from build123d import *

# Parameters (mm, degrees)
SKETCH1_W           = 110
SKETCH1_H           = 70
BOSS_EXTRUDE1_DEPTH = 1
SKETCH2_R           = 5.5
CUT_EXTRUDE1_DEPTH  = 1
CHAMFER1_SIZE       = 5


with BuildPart() as part:
    # Sketch1 → Boss-Extrude1 (new body)
    with BuildSketch(Plane.XY):
        Rectangle(SKETCH1_W, SKETCH1_H)
    extrude(amount=BOSS_EXTRUDE1_DEPTH)

    # Sketch2 → Cut-Extrude1 (cut)
    with BuildSketch(Plane.XY.offset(1)):
        with Locations((-40, 20)):
            Circle(SKETCH2_R)
        with Locations((40, 20)):
            Circle(SKETCH2_R)
        with Locations((-40, -20)):
            Circle(SKETCH2_R)
        with Locations((40, -20)):
            Circle(SKETCH2_R)
    extrude(amount=-CUT_EXTRUDE1_DEPTH, mode=Mode.SUBTRACT)

    # Chamfer1
    chamfer1_edges = [part.edges().sort_by_distance(p)[0] for p in [
        (-55, 35, 0.5),
        (55, 35, 0.5),
        (55, -35, 0.5),
        (-55, -35, 0.5),
    ]]
    chamfer(chamfer1_edges, length=CHAMFER1_SIZE)


solid = part.part
Input: part model. Units: mm. Frame: model coordinates. Coordinates: 2 decimals unless noted, no trailing zeros. Order: outer loops, then holes, each group sorted by start corner. A loop starts at its lowest first (then second) coordinate and runs counter-clockwise, first axis right, second up. Notation, with made-up numbers: M -11,59 L 7,59 A38 cw 7,98 Z; hole C 82.25,84.5 d11. An arc over 180 degrees is marked long. Answer as CSV lines item,"result".
1. Pull-direction query (Y, two-part tool) for faces 1 (the flat face through (-52.5, -32.5, 0.5)), 2 (the flat face through (52.5, 32.5, 0.5)), 3 (the flat face through (-1, 0, 1)), 4 (the cylindrical face through (-45.495, -19.758, 0.507)); classes: released by +Y, released by -Y, zero draft, split by the parting line, or undercut.
Reported:
face 1,"released by -Y"
face 2,"released by +Y"
face 3,"zero draft"
face 4,"undercut"
2. Material intervals for line 1 (Y direction, x = 39.5, z = 0.5); line 2 (X direction, y = -16, z = 0.15); line 3 (X direction, y = 15, z = 0.45), sorted ascending. Write a range as from..to.
Reported:
line 1,"-35..-25.48, -14.52..14.52, 25.48..35"
line 2,"-55..-43.77, -36.23..36.23, 43.77..55"
line 3,"-55..-42.29, -37.71..37.71, 42.29..55"
3. Section A-A (x = 40). Return the cut outline in (y, z).
Reported:
outline,"M -35,0 L -25.5,0 L -25.5,1 L -35,1 Z; M -14.5,0 L 14.5,0 L 14.5,1 L -14.5,1 Z; M 25.5,0 L 35,0 L 35,1 L 25.5,1 Z"
4. Section C-C (y = -20). Return the cut outline in (x, z), then the cut area to 3 significant figures.
Reported:
outline,"M -55,0 L -45.5,0 L -45.5,1 L -55,1 Z; M -34.5,0 L 34.5,0 L 34.5,1 L -34.5,1 Z; M 45.5,0 L 55,0 L 55,1 L 45.5,1 Z"
area,"88.0 mm2"
5. Section B-B (z = 0.3). Return the cut outline in (x, y), then the cut area to 3 significant figures.
Reported:
outline,"M -55,-30 L -50,-35 L 50,-35 L 55,-30 L 55,30 L 50,35 L -50,35 L -55,30 Z; hole C -40,-20 d11; hole C -40,20 d11; hole C 40,-20 d11; hole C 40,20 d11"
area,"7,270 mm2"
